Answer from the drawing. Dimensions are ordinates in mm from the lowest x, y and z of the part. Give positions to 0.01 mm unless a question says otherwise; leave off trailing zeros. Loops run counter-clockwise (first coordinate to the right, second up) from the corner with the lowest first, then second, coordinate; pieces in that order, holes last. Notation, with made-up numbers: (-29, 83) -> (24, 83) arc R25 cw to (24, 113) -> close; hole circle Ø7 at (67, 75.5). An arc over 180 degrees is marked (long way). Return JSON: item names as keys, results as strings. Group by question number.
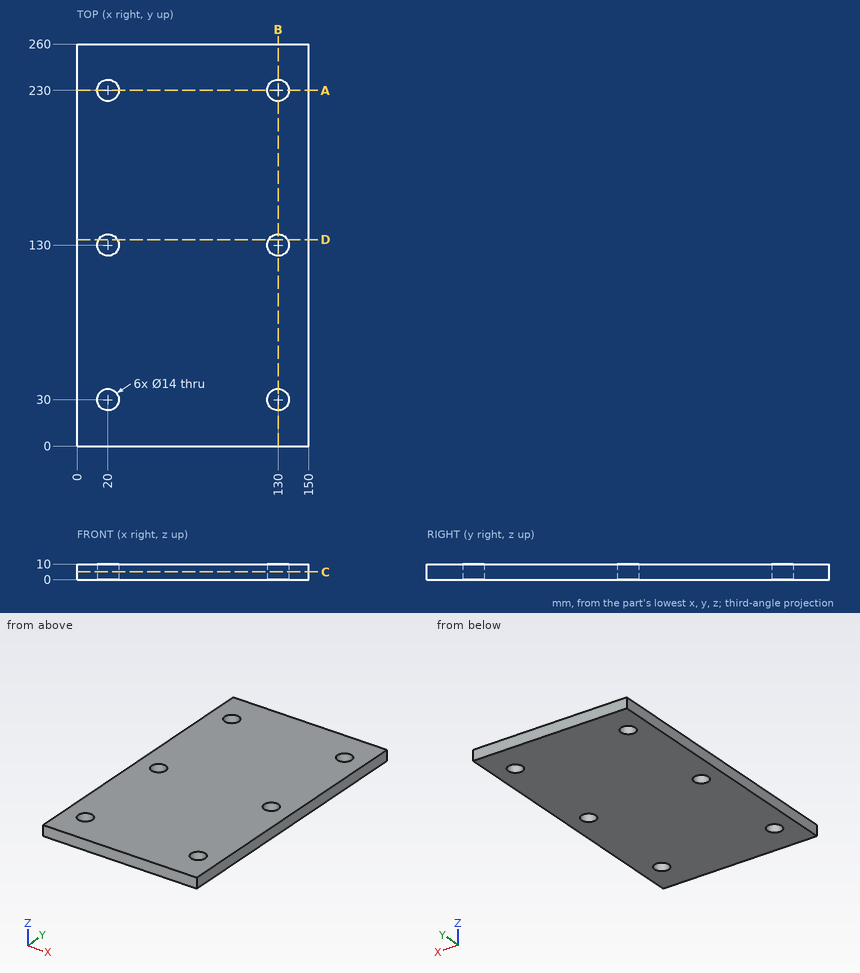
1. Section B-B on x = 130 is taken. Determine the outline of the cut face in (y, z).
2. Section A-A on y = 230 is taken. Determine the outline of the cut face in (x, z), then the cut area to 3 significant figures.
3. A flat-ended cylindrical pin translates along its axis: pin 1 Ø16 at (x, y) = (20, 30) entering from -Z. Find the tip coordinate at first contact, or state that the pin passes through.
4. Section C-C on z = 5 is taken. Determine the outline of the cut face in (x, y).
5. Section D-D on y = 133.5 is taken. Determine the outline of the cut face in (x, z), then the cut area to 3 significant figures.
6. Straight lines are drawn through the part: line 1 (Y direction, x = 20, z = 6.75); line 2 (X direction, y = 232, z = 7.5); line 3 (Y direction, x = 18, z = 7.5). For each, find the intervals that lie inside material, in ascending order. Write a range as from..to.
Completed:
{
 "1": {"outline": "(0, 0) -> (23, 0) -> (23, 10) -> (0, 10) -> close; (37, 0) -> (123, 0) -> (123, 10) -> (37, 10) -> close; (137, 0) -> (223, 0) -> (223, 10) -> (137, 10) -> close; (237, 0) -> (260, 0) -> (260, 10) -> (237, 10) -> close"},
 "2": {"outline": "(0, 0) -> (13, 0) -> (13, 10) -> (0, 10) -> close; (27, 0) -> (123, 0) -> (123, 10) -> (27, 10) -> close; (137, 0) -> (150, 0) -> (150, 10) -> (137, 10) -> close", "area": "1,220 mm²"},
 "3": {"pin 1": "stops at z = 0"},
 "4": {"outline": "(0, 0) -> (150, 0) -> (150, 260) -> (0, 260) -> close; hole circle Ø14 at (20, 30); hole circle Ø14 at (20, 130); hole circle Ø14 at (20, 230); hole circle Ø14 at (130, 30); hole circle Ø14 at (130, 130); hole circle Ø14 at (130, 230)"},
 "5": {"outline": "(0, 0) -> (13.94, 0) -> (13.94, 10) -> (0, 10) -> close; (26.06, 0) -> (123.94, 0) -> (123.94, 10) -> (26.06, 10) -> close; (136.06, 0) -> (150, 0) -> (150, 10) -> (136.06, 10) -> close", "area": "1,260 mm²"},
 "6": {"line 1": "y = 0..23, 37..123, 137..223, 237..260", "line 2": "x = 0..13.29, 26.71..123.29, 136.71..150", "line 3": "y = 0..23.29, 36.71..123.29, 136.71..223.29, 236.71..260"}
}
